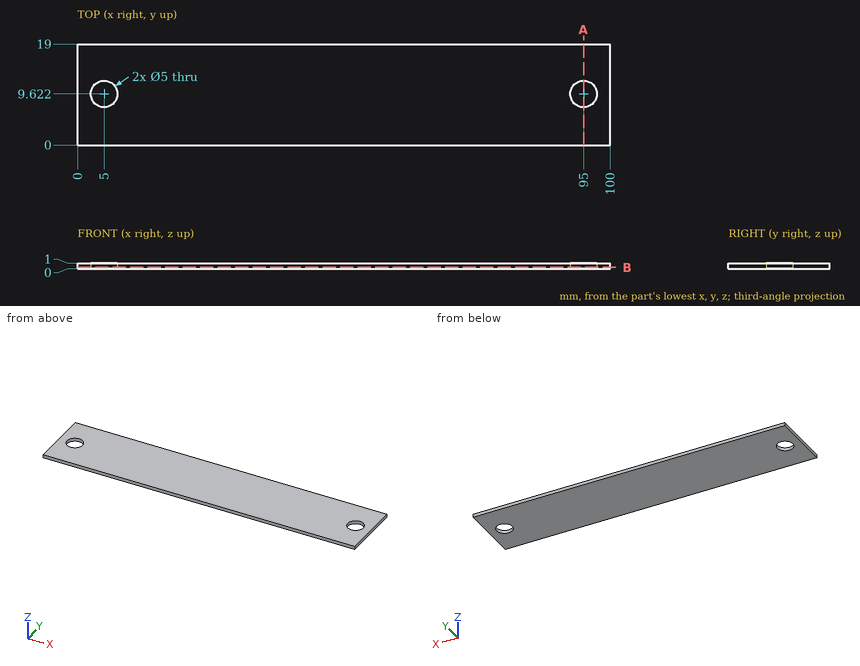
Input: dimensioned drawing with shaded views. Units: mm. Origin: part minimum x, y, z. Round coordinates to 2 decimals unless told otherwise and drop trailing zeros. Order: outer loops, then holes, each group sorted by start corner. A loop starts at its lowest first (then second) coordinate and runs counter-clockwise, first axis right, second up.
Q1. Pin query (flat end, axial travel): pin 1 (8 mm diameter, centred on x = 24, y = 15.5, fed in from -Z); pin 2 (3 mm diameter, centred on x = 95, y = 9.62, fed in from -Z). Return the tip coordinate at first contact, or that it passes through.
Result sheet:
pin 1: stops at z = 0
pin 2: passes through
Q2. Section B-B, the plane z = 0.2. Output: boundary loops of the cut face in (x, y).
Result sheet:
outline: (0, 0) - (100, 0) - (100, 19) - (0, 19) - close; hole circle Ø5 at (5, 9.62); hole circle Ø5 at (95, 9.62)
Q3. Material intervals for probe 1 along Y at (x, z) = (5, 0.45); probe 2 along X at (y, z) = (10.5, 0.35); probe 3 along X at (y, z) = (7.5, 0.95), sorted ascending.
Result sheet:
probe 1: y = 0 to 7.12, 12.12 to 19
probe 2: x = 0 to 2.66, 7.34 to 92.66, 97.34 to 100
probe 3: x = 0 to 3.68, 6.32 to 93.68, 96.32 to 100
Q4. Section A-A, the plane x = 95. Output: boundary loops of the cut face in (y, z), and give its area (3 significant figures).
Result sheet:
outline: (0, 0) - (7.12, 0) - (7.12, 1) - (0, 1) - close; (12.12, 0) - (19, 0) - (19, 1) - (12.12, 1) - close
area: 14.0 mm2
